from build123d import *


with BuildPart() as part:
    # Sketch1 → Revolve1 (revolve)
    with BuildSketch(Plane.XY, mode=Mode.PRIVATE) as revolve1_sk:
        Polygon((-65.629373749, -27.972671928), (-60.629373749, -27.972671928), (-60.629373749, -62.972671928), (-53.129373749, -62.972671928), (-53.129373749, -142.972671928), (-73.129373749, -142.972671928), (-73.129373749, -137.972671928), (-58.129373749, -137.972671928), (-58.129373749, -67.972671928), (-65.629373749, -67.972671928), align=None)
    revolve(revolve1_sk.sketch.rotate(Axis((-73.129373749, -60, 0), (0, -1, 0)), 90), axis=Axis((-73.129373749, -60, 0), (0, -1, 0)))


solid = part.part
Read the model definition and answer for the solid it produces. Units are mm, in the model's axes. A direction names the side the tool comes from. Round coordinates to 2 decimals unless told otherwise and drop trailing zeros. Loops run counter-clockwise (first coordinate to the right, second up) from the corner with the lowest first, then second, coordinate; pieces in that order, holes last.
Q1. Determine the mould class of faces 1 (the face through (-70, -67.973, -7)), 2 (the face through (-73, -142.973, 0)), 3 (the face through (-85.523, -45.718, -1.627)) for opening direction Z: released by +Z, released by -Z, zero draft, split by the parting line, or undercut.
Q2. Section D-D on x = -67.5 is taken. Write down the section's boundary in (y, z).
Q3. Each of these flat-tipped pins is pushed along its axis until it touches: pin 1 (8 mm diameter, centred on y = -56.5, z = 9, fed in from +X); pin 2 (15 mm diameter, centred on x = -69, z = 2.5, fed in from +Y); pin 3 (5 mm diameter, centred on y = -74, z = 15, fed in from -X); pin 4 (12 mm diameter, centred on x = -80, y = -86.5, fed in from +Z). Where does it stop, or does it pass through?
Q4. Consider probe 1 along Y at (x, z) = (-71.5, -11.5); probe 2 along X at (y, z) = (-113, 0); probe 3 along X at (y, z) = (-56, 0). Determine where each line is inside the solid, lowest interval first.
Q5. Section C-C on z = -11 is taken. Write down the section's boundary in (x, y), and give its area (3 significant figures).
Q6. Section A-A on z = 0 is taken. Write down the section's boundary in (x, y).
Q7. Which of the six approach directions +Z, -Z, +X, -X, +Y, -Y give full straight-line access (tool end or side, diameter ignored) to faces 4 (the face through (-73, -137.973, 0)), 5 (the face through (-60, -62.973, 0)), 6 (the face through (-67.7, -27.973, -5.4))?
Q8. Section B-B on x = -84 is taken. Write down the section's boundary in (y, z), and give its area (3 significant figures).
Output:
1. face 1: undercut
1. face 2: zero draft
1. face 3: split by the parting line
2. outline: (-142.97, -19.19) - (-62.97, -19.19) - (-62.97, -11.16) - (-27.97, -11.16) - (-27.97, -4.96) - (-67.97, -4.96) - (-67.97, -13.9) - (-137.97, -13.9) - (-137.97, 13.9) - (-67.97, 13.9) - (-67.97, 4.96) - (-27.97, 4.96) - (-27.97, 11.16) - (-62.97, 11.16) - (-62.97, 19.19) - (-142.97, 19.19) - close
3. pin 1: stops at x = -61.67
3. pin 2: stops at y = -27.97
3. pin 3: stops at x = -88.74
3. pin 4: stops at z = 19.98
4. probe 1: y = -142.97 to -137.97, -67.97 to -27.97
4. probe 2: x = -93.13 to -88.13, -58.13 to -53.13
4. probe 3: x = -85.63 to -80.63, -65.63 to -60.63
5. outline: (-89.83, -142.97) - (-56.43, -142.97) - (-56.43, -62.97) - (-67.19, -62.97) - (-67.19, -27.97) - (-79.07, -27.97) - (-79.07, -62.97) - (-89.83, -62.97) - close; hole (-83.33, -137.97) - (-62.93, -137.97) - (-62.93, -67.97) - (-83.33, -67.97) - close
5. area: 1,660 mm2
6. outline: (-93.13, -142.97) - (-53.13, -142.97) - (-53.13, -62.97) - (-60.63, -62.97) - (-60.63, -27.97) - (-65.63, -27.97) - (-65.63, -67.97) - (-58.13, -67.97) - (-58.13, -137.97) - (-88.13, -137.97) - (-88.13, -67.97) - (-80.63, -67.97) - (-80.63, -27.97) - (-85.63, -27.97) - (-85.63, -62.97) - (-93.13, -62.97) - close
7. face 4: none
7. face 5: +Y
7. face 6: +Z, -Z, +X, -X, +Y
8. outline: (-142.97, -16.79) - (-62.97, -16.79) - (-62.97, -6.17) - (-27.97, -6.17) - (-27.97, 6.17) - (-62.97, 6.17) - (-62.97, 16.79) - (-142.97, 16.79) - close; hole (-137.97, -10.34) - (-67.97, -10.34) - (-67.97, 10.34) - (-137.97, 10.34) - close
8. area: 1,670 mm2
